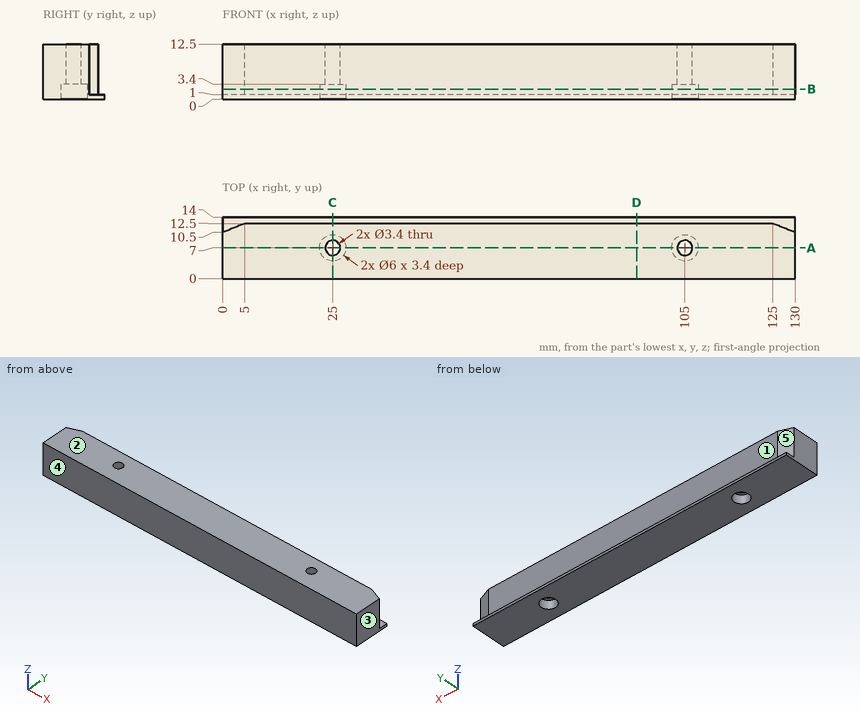
Verification items for this drawing (mm, ordinates from the low corner). A direction names the side the tool comes from. Give positions to 0.01 mm unless a question says otherwise; leave off trailing zeros. Write each loop counter-clockwise with the first axis right and the second up, starting at its lowest first coordinate (ties: lowest second). Pieces come first, ordered by that corner, then holes. Notation, with made-up numbers: (23, 30.5) - (80, 30.5) arc R19 cw to (80, 45.5) - close; hole circle Ø2 at (-32, -17). An arc over 180 degrees is marked (long way). Answer as CSV lines item,"result". Start each with the question number.
1. Sectioned sample at C-C (x = 25). Record the boundary of the cut face in (y, z).
2. Sectioned sample at D-D (x = 94). Record the boundary of the cut face in (y, z), then the cut area to 3 significant figures.
3. Draft check along X on the marked faces 3, 4 and 5. Enter one of: pulls with the +X half, pulls with the -X half, needs draft (parallel to the pull), parting line crosses it, or undercut.
4. Sectioned sample at A-A (y = 7). Record the boundary of the cut face in (x, z).
5. Thickness scan on line 1 (X direction, y = 9.25, z = 2.5); line 2 (X direction, y = 7.5, z = 7.25); line 3 (Y direction, x = 25, z = 1.2). Record the ranges inside material, lowest first.
6. Depth check by flat-ended pin: pin 1 (6 mm diameter, centred on x = 91.5, z = 9, fed in from +Y); pin 2 (5 mm diameter, centred on x = 105, y = 7, fed in from -Z). Enter the tip coordinate at first touch or a pass-through.
7. Set-up check for the marked faces 1 and 2: record each of +Z, -Z, +X, -X, +Y, -Y from which the full face is reachable in a straight line by a thin tool's end or side.
8. Sectioned sample at B-B (z = 2.25). Record the boundary of the cut face in (x, y), then the cut area to 3 significant figures.
Derived:
1,outline,"(0, 0) - (4, 0) - (4, 3.4) - (5.3, 3.4) - (5.3, 12.5) - (0, 12.5) - close; (8.7, 3.4) - (10, 3.4) - (10, 0) - (14, 0) - (14, 1) - (12.5, 1) - (12.5, 12.5) - (8.7, 12.5) - close"
2,outline,"(0, 0) - (14, 0) - (14, 1) - (12.5, 1) - (12.5, 12.5) - (0, 12.5) - close"
2,area,"158 mm²"
3,face 3,"pulls with the +X half"
3,face 4,"needs draft"
3,face 5,"pulls with the -X half"
4,outline,"(0, 0) - (22, 0) - (22, 3.4) - (23.3, 3.4) - (23.3, 12.5) - (0, 12.5) - close; (26.7, 3.4) - (28, 3.4) - (28, 0) - (102, 0) - (102, 3.4) - (103.3, 3.4) - (103.3, 12.5) - (26.7, 12.5) - close; (106.7, 3.4) - (108, 3.4) - (108, 0) - (130, 0) - (130, 12.5) - (106.7, 12.5) - close"
5,line 1,"0 to 23.02, 26.98 to 103.02, 106.98 to 130"
5,line 2,"0 to 23.38, 26.62 to 103.38, 106.62 to 130"
5,line 3,"0 to 4, 10 to 12.5"
6,pin 1,"y = 12.5"
6,pin 2,"z = 3.4"
7,face 1,"+Z, +X, -X, +Y"
7,face 2,"+Z, +X, -X, +Y, -Y"
8,outline,"(0, 0) - (130, 0) - (130, 10.5) - (125, 12.5) - (5, 12.5) - (0, 10.5) - close; hole circle Ø6 at (25, 7); hole circle Ø6 at (105, 7)"
8,area,"1,560 mm²"
